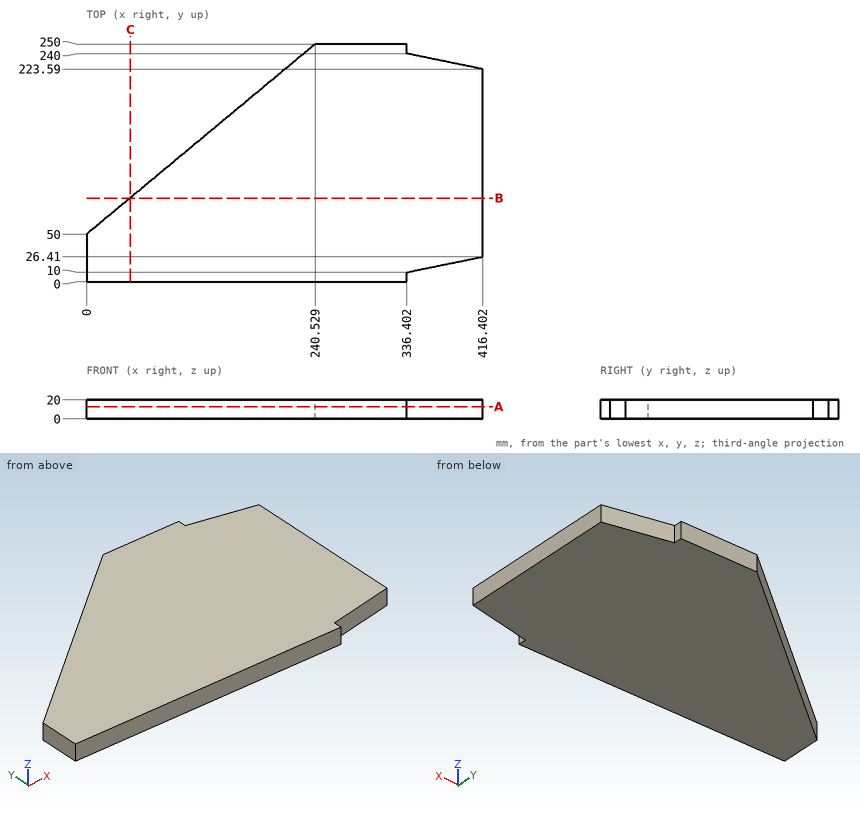
Geometry: see drawing. Coordinates: mm, zero at the bounding-box minimum. Give positions to 0.01 mm unless a question says otherwise; leave off trailing zeros. Write each loop counter-clockwise with the first axis right and the second up, starting at its lowest first coordinate (ties: lowest second). Pieces come first, ordered by that corner, then holes. Notation, with made-up numbers: M 51,53 L 104,53 A15 ccw 104,60 Z; hole C -31,10 d4. An arc over 180 degrees is marked long. Answer in a Markdown table with one row per item. Add a question column.
(1) First-contact query: pin 1 (3 mm diameter, centred on y = 116.5, z = 8.5, fed in from -X); pin 2 (6 mm diameter, centred on x = 166, z = 16.5, fed in from +Y) (1 decimal); pin 3 (11 mm diameter, centred on y = 4, z = 8, fed in from +X). Flat tips, straight axial feed; report the tip coordinate or a pass-through.
(2) Ray query, line 1 (Y direction, x = 219, z = 3.75); line 2 (Y direction, x = 33.5, z = 10.75) (1 decimal); line 3 (X direction, y = 172.5, z = 9) (1 decimal). Return the intervals inside material, ascending.
(3) Section B-B on y = 88. Return loops of the section in (x, z).
(4) Section C-C on x = 46. Return loops of the section in (y, z), and give its area (4 significant figures).
(5) Section A-A on z = 12.75. Return loops of the section in (x, y).
Result set:
| question | item | result |
|---|---|---|
| 1 | pin 1 | stops at x = 78.17 |
| 1 | pin 2 | stops at y = 190.5 |
| 1 | pin 3 | stops at x = 336.4 |
| 2 | line 1 | y = 0 to 232.1 |
| 2 | line 2 | y = 0 to 77.9 |
| 2 | line 3 | x = 147.3 to 416.4 |
| 3 | outline | M 45.7,0 L 416.4,0 L 416.4,20 L 45.7,20 Z |
| 4 | outline | M 0,0 L 88.25,0 L 88.25,20 L 0,20 Z |
| 4 | area | 1,765 mm^2 |
| 5 | outline | M 0,0 L 336.4,0 L 336.4,10 L 416.4,26.41 L 416.4,223.59 L 336.4,240 L 336.4,250 L 240.53,250 L 0,50 Z |
